from build123d import *

# Parameters (mm, degrees)
BOSS_EXTRUDE1_DEPTH    = 15
M24_TAPPED_HOLE1_D     = 21
M24_TAPPED_HOLE1_DEPTH = 57
M24_TAPPED_HOLE1_TIP   = 6.3090365


with BuildPart() as part:
    # Sketch1 → Boss-Extrude1 (new body)
    with BuildSketch(Plane.XY):
        Polygon((18.475208614, 0), (9.237604307, 16), (-9.237604307, 16), (-18.475208614, 0), (-9.237604307, -16), (9.237604307, -16), align=None)
    extrude(amount=BOSS_EXTRUDE1_DEPTH)

    # M24 Tapped Hole1
    with Locations(Plane.XY.offset(15)):
        with Locations((0, 0)):
            Hole(M24_TAPPED_HOLE1_D / 2, depth=M24_TAPPED_HOLE1_DEPTH)
            with Locations((0, 0, -(M24_TAPPED_HOLE1_DEPTH + M24_TAPPED_HOLE1_TIP / 2))):  # 118° drill point
                Cone(0, M24_TAPPED_HOLE1_D / 2, M24_TAPPED_HOLE1_TIP, mode=Mode.SUBTRACT)


solid = part.part
For this review, take the finished solid that the model builds, in its own axes (mm). Give positions to 0.01 mm unless a question says otherwise; leave off trailing zeros. Loops run counter-clockwise (first coordinate to the right, second up) from the corner with the lowest first, then second, coordinate; pieces in that order, holes last.
Item 1: For line 1 along Y through (x, z) = (0, 11.5); line 2 along X through (y, z) = (5, 9.25); line 3 along X through (y, z) = (1, 12), list the stretches that pass through material, from the lowest coordinate up.
Item 2: Insertion check: pin 1 (12 mm diameter, centred on x = 1, y = 2.5, fed in from -Z); pin 2 (1.5 mm diameter, centred on y = 5, z = 3, fed in from -X); pin 3 (12 mm diameter, centred on x = 2.5, y = -12, fed in from -Z); pin 4 (3 mm diameter, centred on y = 10, z = 9, fed in from -X). Each pin has a flat end and moves straight along its axis. Give the tip position at first contact, or say it passes through.
Item 3: Take a section at C-C, the plane z = 3. State the section outline as (x, y) points, and give its area (3 significant figures).
Item 4: Take a section at A-A, the plane x = 0. State the section outline as (y, z) points, and give its area (3 significant figures).
Item 5: Draft analysis for pull direction Y (two halves, no side actions). For faces 1 (the flat face through (-13.8, 8.1, 7.4)), 2 (the flat face through (8, 7.3, 15)), 3 (the cylindrical face through (-10, 3.2, 7.4)), state which applies: +Y half, -Y half, draft (parallel to the pull), parting line (faces both ways), or undercut.
Item 6: Take a section at B-B, the plane y = -1. State the section outline as (x, z) points, and give its area (3 significant figures).
Item 7: Take a section at D-D, the plane y = 13.5. State the section outline as (x, z) points.
Calculated:
1. line 1: y = -16 to -10.5, 10.5 to 16
1. line 2: x = -15.59 to -9.23, 9.23 to 15.59
1. line 3: x = -17.9 to -10.45, 10.45 to 17.9
2. pin 1: passes through
2. pin 2: stops at x = -16.02
2. pin 3: stops at z = 0
2. pin 4: stops at x = -13.57
3. outline: (-18.48, 0) - (-9.24, -16) - (9.24, -16) - (18.48, 0) - (9.24, 16) - (-9.24, 16) - close; hole circle Ø21 at (0, 0)
3. area: 540 mm2
4. outline: (-16, 0) - (-10.5, 0) - (-10.5, 15) - (-16, 15) - close; (10.5, 0) - (16, 0) - (16, 15) - (10.5, 15) - close
4. area: 165 mm2
5. face 1: +Y half
5. face 2: draft
5. face 3: undercut
6. outline: (-17.9, 0) - (-10.45, 0) - (-10.45, 15) - (-17.9, 15) - close; (10.45, 0) - (17.9, 0) - (17.9, 15) - (10.45, 15) - close
6. area: 223 mm2
7. outline: (-10.68, 0) - (10.68, 0) - (10.68, 15) - (-10.68, 15) - close
